For this review, use the dimensioned drawing (mm, ordinates from the lowest corner) and the shaded views. A direction names the side the tool comes from. Round coordinates to 2 decimals unless told otherwise and drop trailing zeros. Loops run counter-clockwise (first coordinate to the right, second up) from the corner with the lowest first, then second, coordinate; pieces in that order, holes last. Notation, with made-up numbers: M -14,-7.5 L 16,-7.5 A7 cw 16,-0.5 Z; hole C -36.5,15.5 d11. An arc over 180 degrees is marked long. Use a Markdown table: item, result. Add a question column.
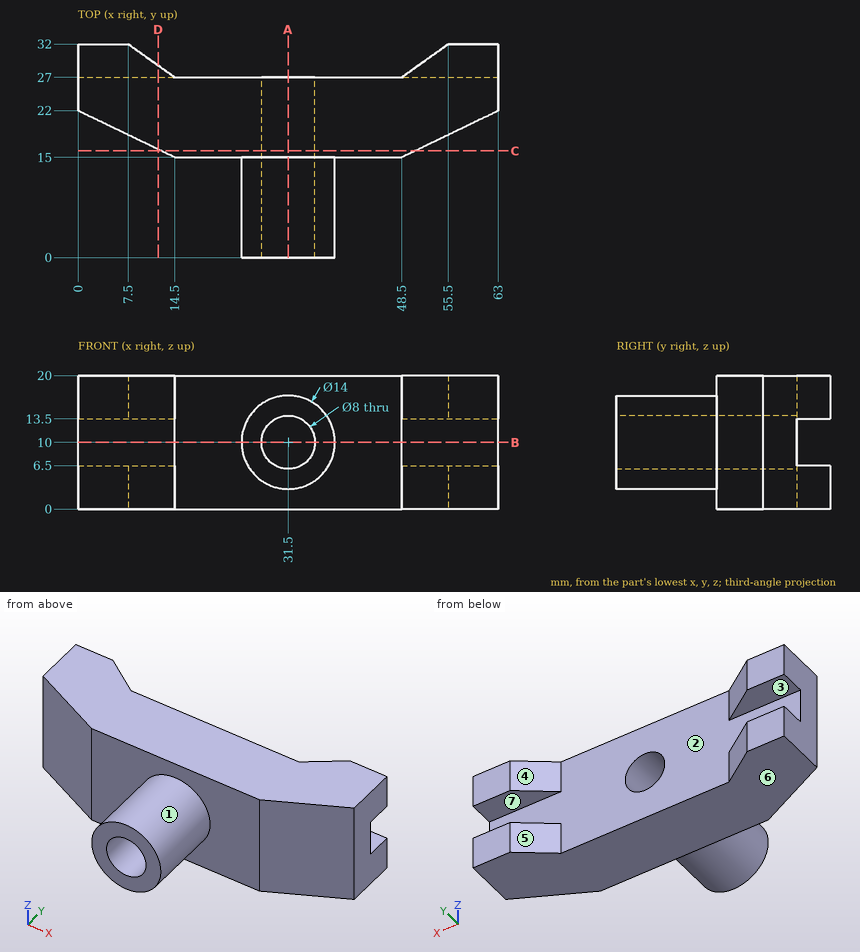
(1) Consider section B-B, the plane z = 10. Give the boundary of the cut face in (x, y).
(2) To check wall thickness, follow probe 1 along X at (y, z) = (14, 10); probe 2 along Y at (x, z) = (35, 4.5); probe 3 along X at (y, z) = (17, 10). State the ranges of each line that lie inside material, in increasing order.
(3) Consider section C-C, the plane y = 16. Give the boundary of the cut face in (x, z), then the cut area to 3 significant figures.
(4) Consider section D-D, the plane x = 12. Give the boundary of the cut face in (y, z), then the cut area to 3 significant figures.
(5) Consider section A-A, the plane x = 31.5. Give the boundary of the cut face in (y, z), then the cut area to 3 significant figures.
(6) Insertion check: pin 1 Ø10 at (x, z) = (29.5, 9.5) entering from -Y; pin 2 Ø5 at (x, z) = (32, 11.5) entering from +Y; pin 3 Ø1.5 at (y, z) = (14, 7) entering from +X; pin 4 Ø8 at (y, z) = (15, 11.5) entering from +X. Each pin has a flat end and moves straight along its axis. Give the tip position at first contact, or say it passes through.
(7) For the marked faces 1, 2, 3 and 4, list the 3-axis set-ups (+Z, -Z, +X, -X, +Y, -Y) from which the entire face can be reached by the end or side of a thin tool; tool diameter is ignored.
(8) Draft analysis for pull direction Z (two halves, no side actions). For the marked faces 5, 6 and 7, state which applies: released by +Z, released by -Z, zero draft, split by the parting line, or undercut.
Found:
| question | item | result |
|---|---|---|
| 1 | outline | M 0,22 L 14.5,15 L 24.5,15 L 24.5,0 L 27.5,0 L 27.5,27 L 0,27 Z; M 35.5,0 L 38.5,0 L 38.5,15 L 48.5,15 L 63,22 L 63,27 L 35.5,27 Z |
| 2 | probe 1 | x = 24.5 to 27.5, 35.5 to 38.5 |
| 2 | probe 2 | y = 0 to 27 |
| 2 | probe 3 | x = 10.36 to 27.5, 35.5 to 52.64 |
| 3 | outline | M 12.43,0 L 50.57,0 L 50.57,20 L 12.43,20 Z; hole C 31.5,10 d8 |
| 3 | area | 713 mm^2 |
| 4 | outline | M 16.21,0 L 28.79,0 L 28.79,6.5 L 27,6.5 L 27,13.5 L 28.79,13.5 L 28.79,20 L 16.21,20 Z |
| 4 | area | 239 mm^2 |
| 5 | outline | M 0,3 L 15,3 L 15,0 L 27,0 L 27,6 L 0,6 Z; M 0,14 L 27,14 L 27,20 L 15,20 L 15,17 L 0,17 Z |
| 5 | area | 234 mm^2 |
| 6 | pin 1 | stops at y = 0 |
| 6 | pin 2 | stops at y = 27 |
| 6 | pin 3 | stops at x = 38.13 |
| 6 | pin 4 | stops at x = 56.79 |
| 7 | face 1 | -Y |
| 7 | face 2 | +Y |
| 7 | face 3 | +X, -X, +Y |
| 7 | face 4 | +Z, -Z, +Y |
| 8 | face 5 | zero draft |
| 8 | face 6 | released by -Z |
| 8 | face 7 | undercut |
